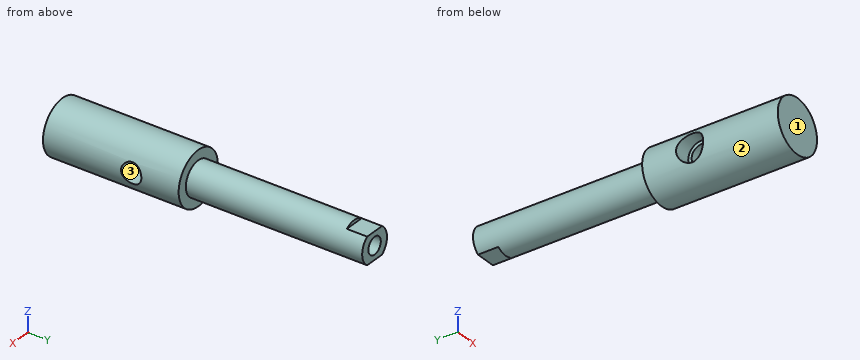
```python
from build123d import *

# Parameters (mm, degrees)
SKETCH1_R               = 3.95
BOSS_EXTRUDE1_DEPTH     = 20
SKETCH2_R               = 2.5
BOSS_EXTRUDE2_DEPTH     = 26
SKETCH3_OUTSIDE_W       = 19.368
SKETCH3_OUTSIDE_H       = 19.368
SKETCH3_OUTSIDE_W_2     = 5.796030148
SKETCH3_OUTSIDE_H_2     = 4
CUT_EXTRUDE1_DEPTH      = 3
CUT_EXTRUDE2_DEPTH      = 47.337943416
CUT_EXTRUDE2_DEPTH_BACK = 47.337943416
SKETCH4_R               = 1.5
CUT_EXTRUDE3_START      = -1.5
SKETCH5_R               = 2
CUT_EXTRUDE3_DEPTH      = 10


with BuildPart() as part:
    # Sketch1 → Boss-Extrude1 (new body)
    with BuildSketch(Plane(origin=(0, 0, 0), x_dir=(1, 0, 0), z_dir=(0, 1, 0))):
        with Locations(Location((0, 0, 0), (0, 0, 270))):
            Circle(SKETCH1_R)
    extrude(amount=BOSS_EXTRUDE1_DEPTH)

    # Sketch2 → Boss-Extrude2 (add)
    with BuildSketch(Plane(origin=(0, 20, 0), x_dir=(1, 0, 0), z_dir=(0, 1, 0))):
        with Locations(Location((0, 0, 0), (0, 0, 90))):
            Circle(SKETCH2_R)
    extrude(amount=BOSS_EXTRUDE2_DEPTH)

    # Sketch3 outside → Cut-Extrude1 (cut)
    with BuildSketch(Plane(origin=(0, 46, 0), x_dir=(1, 0, 0), z_dir=(0, 1, 0))):
        Rectangle(SKETCH3_OUTSIDE_W, SKETCH3_OUTSIDE_H)
        Rectangle(SKETCH3_OUTSIDE_W_2, SKETCH3_OUTSIDE_H_2, mode=Mode.SUBTRACT)
    extrude(amount=-CUT_EXTRUDE1_DEPTH, mode=Mode.SUBTRACT)

    # Sketch4 → Cut-Extrude2 (cut, two sides: drawn at the far end of the back side and taken through both)
    with BuildSketch(Plane(origin=(0, 0, 0), x_dir=(0, 0, -1), z_dir=(1, 0, 0)).offset(-CUT_EXTRUDE2_DEPTH_BACK)):
        with Locations((0, 13)):
            Circle(SKETCH4_R)
    extrude(amount=CUT_EXTRUDE2_DEPTH + CUT_EXTRUDE2_DEPTH_BACK, mode=Mode.SUBTRACT)

    # Sketch5 → Cut-Extrude3 (cut)
    with BuildSketch(Plane(origin=(0, 0, 0), x_dir=(0, 0, -1), z_dir=(1, 0, 0)).offset(CUT_EXTRUDE3_START)):
        with Locations((0, 13)):
            Circle(SKETCH5_R)
    extrude(amount=-CUT_EXTRUDE3_DEPTH, mode=Mode.SUBTRACT)

    # Sketch6 → M3 Tapped Hole2 (revolve, cut)
    with BuildSketch(Plane(origin=(0, 46, 0), x_dir=(0, 0, 1), z_dir=(1, 0, 0))):
        Polygon((0, 0), (0, 8.251075774), (1.25, 7.5), (1.25, 0), align=None)
    revolve(axis=Axis((0, 52.35, 0), (0, -1, 0)), mode=Mode.SUBTRACT)


solid = part.part
```
Geometry check sheet. Reference: the model listing, model coordinates, mm. Face numbers are marked on the shaded views. Round coordinates to 2 decimals unless told otherwise and drop trailing zeros. Order: outer loops, then holes, each group sorted by start corner. A loop starts at its lowest first (then second) coordinate and runs counter-clockwise, first axis right, second up. Notation, with made-up numbers: M -23,-10 L -8,-10 A28 ccw -8,18 Z; hole C -3.5,64 d1. An arc over 180 degrees is marked long. Write item = value, one per line.
Q1. Scan lines: line 1 (Y direction, x = -2.2, z = 0); line 2 (X direction, y = 39, z = 0); line 3 (Y direction, x = -3, z = 0). Record each from-to range of solid material in increasing order.
Answer block:
line_1 = 0 to 11, 15 to 46
line_2 = -2.5 to -1.25, 1.25 to 2.5
line_3 = 0 to 11, 15 to 20
Q2. Section check A-A (y = 14). Enter the section's corners in (x, z), plus the area to 3 significant figures.
Answer block:
outline = M -3.55,-1.73 A3.95 ccw 3.79,-1.12 L -1.5,-1.12 L -1.5,-1.73 Z; M -3.55,1.73 L -1.5,1.73 L -1.5,1.12 L 3.79,1.12 A3.95 ccw Z
area = 28.9 mm^2
Q3. Release check for a two-part mould opening along Z. For the marked faces 1, 2 and 3 record: released by +Z, released by -Z, zero draft, split by the parting line, or undercut.
Answer block:
face_1 = zero draft
face_2 = split by the parting line
face_3 = undercut
Q4. Section check B-B (y = 22). Enter the section's corners in (x, z), plus the area to 3 significant figures.
Answer block:
outline = C 0,0 d5
area = 19.6 mm^2
Q5. Depth check by flat-ended pin: pin 1 Ø1 at (x, y) = (-0.5, 38) entering from -Z; pin 2 Ø1.5 at (x, z) = (0, 2.5) entering from -Y; pin 3 Ø0.9 at (x, y) = (0, 45) entering from -Z; pin 4 Ø2.5 at (y, z) = (13, 0) entering from +X. Enter the tip coordinate at first touch or a pass-through.
Answer block:
pin_1 = -2.5
pin_2 = 0
pin_3 = -2
pin_4 = through
